```python
from build123d import *

# Parameters (mm, degrees)
SKETCH1_R           = 3.5
BOSS_EXTRUDE1_DEPTH = 8


with BuildPart() as part:
    # Sketch1 → Boss-Extrude1 (new body)
    with BuildSketch(Plane.XY):
        with BuildLine():
            Line((0, 8), (22, 8))
            Line((22, 8), (22, -8))
            Line((22, -8), (0, -8))
            ThreePointArc((0, -8), (-8, 0), (0, 8))
        make_face()
        Circle(SKETCH1_R, mode=Mode.SUBTRACT)
    extrude(amount=BOSS_EXTRUDE1_DEPTH)


solid = part.part
```
Build history of the part. All positions in model axes, mm. Coordinates: 2 decimals unless noted, no trailing zeros. Order: outer loops, then holes, each group sorted by start corner. A loop starts at its lowest first (then second) coordinate and runs counter-clockwise, first axis right, second up.
Item 1: Saw through at C-C on z = 6.5. List the corners of the cut face in (x, y).
Filled in:
outline: (0, -8) - (22, -8) - (22, 8) - (0, 8) arc R8 ccw to start; hole circle Ø7 at (0, 0)
Item 2: Drill centre lines: L1, parallel to Y at x = 0, z = 4; L2, parallel to X at y = -2, z = 7.75; L3, parallel to X at y = -1.75, z = 5. Where is each one in solid material? Low to high.
Filled in:
L1: y = -8 to -3.5, 3.5 to 8
L2: x = -7.75 to -2.87, 2.87 to 22
L3: x = -7.81 to -3.03, 3.03 to 22
Item 3: Saw through at A-A on y = 0. List the corners of the cut face in (x, z).
Filled in:
outline: (-8, 0) - (-3.5, 0) - (-3.5, 8) - (-8, 8) - close; (3.5, 0) - (22, 0) - (22, 8) - (3.5, 8) - close
Item 4: Saw through at B-B on x = 0.75. List the corners of the cut face in (y, z).
Filled in:
outline: (-8, 0) - (-3.42, 0) - (-3.42, 8) - (-8, 8) - close; (3.42, 0) - (8, 0) - (8, 8) - (3.42, 8) - close
Item 5: Drop a flat-ended pin along its axis: pin 1 Ø1 at (y, z) = (-5.5, 2.5) entering from -X (3 decimals). Give the stop position or say it passes through.
Filled in:
pin 1: stops at x = -6.245
Item 6: Saw through at D-D on y = -4.25. List the corners of the cut face in (x, z).
Filled in:
outline: (-6.78, 0) - (22, 0) - (22, 8) - (-6.78, 8) - close
Item 7: Mould opens along X. For faces 1 (the cylindrical face through (3.233, -1.341, 3.944)), 2 (the cylindrical face through (-8, 0, 4)), 3 (the flat face through (22, 0, 4)) say: released by +X, released by -X, zero draft, split by the parting line, or undercut.
Filled in:
face 1: undercut
face 2: released by -X
face 3: released by +X
